```python
from build123d import *

# Parameters (mm, degrees)
SKETCH1_W           = 114
SKETCH1_H           = 114
SKETCH1_R           = 28.25
BOSS_EXTRUDE1_DEPTH = 28
FILLET1_R           = 3
FILLET3_R           = 34


with BuildPart() as part:
    # Sketch1 → Boss-Extrude1 (new body)
    with BuildSketch(Plane.XY):
        Rectangle(SKETCH1_W, SKETCH1_H)
        Circle(SKETCH1_R, mode=Mode.SUBTRACT)
    extrude(amount=BOSS_EXTRUDE1_DEPTH)

    # Fillet1
    fillet1_edges = [part.edges().sort_by_distance(p)[0] for p in [
        (-28.25, 0, 0),
        (-28.25, 0, 28),
    ]]
    fillet(fillet1_edges, radius=FILLET1_R)

    # Fillet3
    fillet3_edges = [part.edges().sort_by_distance(p)[0] for p in [
        (-57, 57, 14),
        (57, -57, 14),
    ]]
    fillet(fillet3_edges, radius=FILLET3_R)


solid = part.part
```
Read the model definition and answer for the solid it produces. Units are mm, in the model's axes. Give positions to 0.01 mm unless a question says otherwise; leave off trailing zeros. Write each loop counter-clockwise with the first axis right and the second up, starting at its lowest first coordinate (ties: lowest second). Pieces come first, ordered by that corner, then holes. Notation, with made-up numbers: (1, -16) -> (19, -16) arc R34 cw to (19, 21) -> close; hole circle Ø9 at (-38.5, 29.25). An arc over 180 degrees is marked (long way). Answer in a Markdown table with one row per item.
1) Section A-A on y = 0 is taken. Give the vertices of the cut face in (x, z), plus the area to 3 significant figures.
Results list:
| item | result |
|---|---|
| outline | (-57, 0) -> (-31.25, 0) arc R3 ccw to (-28.25, 3) -> (-28.25, 25) arc R3 ccw to (-31.25, 28) -> (-57, 28) -> close; (28.25, 3) arc R3 ccw to (31.25, 0) -> (57, 0) -> (57, 28) -> (31.25, 28) arc R3 ccw to (28.25, 25) -> close |
| area | 1,600 mm^2 |
2) Section D-D on x = 34.5 is taken. Give the vertices of the cut face in (y, z).
Results list:
| item | result |
|---|---|
| outline | (-55, 0) -> (57, 0) -> (57, 28) -> (-55, 28) -> close |
3) Section B-B on z = 19.25 is taken. Give the vertices of the cut face in (x, y), plus the area to 3 significant figures.
Results list:
| item | result |
|---|---|
| outline | (-57, -57) -> (23, -57) arc R34 ccw to (57, -23) -> (57, 57) -> (-23, 57) arc R34 ccw to (-57, 23) -> close; hole circle Ø56.5 at (0, 0) |
| area | 9,990 mm^2 |
4) Determine the mould class of faces 1 (the cylindrical face through (15.19, 23.82, 13.85)), 2 (the flat face through (-26, 26, 0)), 3 (the flat face through (-18, -57, 14)), 4 (the flat face through (16, 57, 14)) for opening direction Y: released by +Y, released by -Y, zero draft, split by the parting line, or undercut.
Results list:
| item | result |
|---|---|
| face 1 | undercut |
| face 2 | zero draft |
| face 3 | released by -Y |
| face 4 | released by +Y |
5) Each of these flat-tipped pins is pushed along its axis until it touches: pin 1 Ø1.5 at (x, z) = (-27, 24) entering from +Y; pin 2 Ø8 at (x, y) = (37.5, -9) entering from -Z; pin 3 Ø1.5 at (x, z) = (34, 24.5) entering from -Y. Where does it stop, or does it pass through?
Results list:
| item | result |
|---|---|
| pin 1 | y = 56.84 |
| pin 2 | z = 0 |
| pin 3 | y = -55.42 |
6) Straight lines are drawn through the part: line 1 (Y direction, x = 0, z = 16); line 2 (X direction, y = 25.5, z = 19.25); line 3 (X direction, y = 4.5, z = 10.25). For each, find the intervals that lie inside material, in ascending order. Write a range as [from, to].
Results list:
| item | result |
|---|---|
| line 1 | [-57, -28.25], [28.25, 57] |
| line 2 | [-56.91, -12.16], [12.16, 57] |
| line 3 | [-57, -27.89], [27.89, 57] |
